from build123d import *

# Parameters (mm, degrees)
SKETCH2_W               = 6
SKETCH2_H               = 15
CUT_EXTRUDE1_DEPTH      = 45.71
CUT_EXTRUDE2_DEPTH      = 57.171431365
CUT_EXTRUDE2_DEPTH_BACK = 19
SKETCH4_R               = 3


with BuildPart() as part:
    # Model → Revolve1 (revolve)
    with BuildSketch(Plane.XY, mode=Mode.PRIVATE) as revolve1_sk:
        with BuildLine():
            Line((-27.291095715, -5.663546948), (-27.291095715, -10.663546948))
            Line((-27.291095715, -10.663546948), (-27.291095715, -51.373546948))
            ThreePointArc((-27.291095715, -51.373546948), (-28.755561809, -54.909080854), (-32.291095715, -56.373546948))
            Line((-32.291095715, -56.373546948), (-32.291095715, -52.264917369))
            Line((-32.291095715, -52.264917369), (-32.291095715, -10.663546948))
            Line((-32.291095715, -10.663546948), (-32.291095715, 35.040839423))
            Line((-32.291095715, 35.040839423), (-30.291095715, 35.040839423))
            Line((-30.291095715, 35.040839423), (-30.291095715, 26.12431753))
            Line((-30.291095715, 26.12431753), (-28.291095715, 26.12431753))
            Line((-28.291095715, 26.12431753), (-28.291095715, 5.494079969))
            Line((-28.291095715, 5.494079969), (-27.291095715, 5.494079969))
            Line((-27.291095715, 5.494079969), (-27.291095715, 2.336453052))
            Line((-27.291095715, 2.336453052), (-28.291095714, 2.336453052))
            Line((-28.291095714, 2.336453052), (-28.291095714, -5.663546948))
            Line((-28.291095714, -5.663546948), (-27.291095715, -5.663546948))
        make_face()
    revolve(revolve1_sk.sketch.rotate(Axis((-32.291095715, 35.040839423, 0), (0, 1, 0)), 90), axis=Axis((-32.291095715, 35.040839423, 0), (0, 1, 0)))

    # Sketch2 → Cut-Extrude1 (cut)
    with BuildSketch(Plane(origin=(0, -56.373546948, 0), x_dir=(-1, 0, 0), z_dir=(0, -1, 0))):
        with Locations((32.291095715, 1.617056414)):
            Rectangle(SKETCH2_W, SKETCH2_H)
    extrude(amount=-CUT_EXTRUDE1_DEPTH, mode=Mode.SUBTRACT)

    # Sketch4 → Cut-Extrude2 (cut, two sides: drawn at the far end of the back side and taken through both)
    with BuildSketch(Plane(origin=(-35.291095715, 0, 0), x_dir=(0, 0, -1), z_dir=(1, 0, 0)).offset(-CUT_EXTRUDE2_DEPTH_BACK)):
        with Locations(Location((0, -51.373546948, 0), (0, 0, 180))):
            Circle(SKETCH4_R)
    extrude(amount=CUT_EXTRUDE2_DEPTH + CUT_EXTRUDE2_DEPTH_BACK, mode=Mode.SUBTRACT)


solid = part.part
Verification items for the finished model (mm, model axes). A direction names the side the tool comes from. Round coordinates to 2 decimals unless told otherwise and drop trailing zeros. Loops run counter-clockwise (first coordinate to the right, second up) from the corner with the lowest first, then second, coordinate; pieces in that order, holes last. Notation, with made-up numbers: (-19.75, 27) - (12.25, 27) arc R27 ccw to (12.25, 64) - close; hole circle Ø8 at (59.5, 88). An arc over 180 degrees is marked (long way). Answer in a Markdown table with one row per item. Add a question column.
Q1. Section check B-B on y = 1. Enter the section's corners in (x, z), plus the area to 3 significant figures.
Q2. Release check for a two-part mould opening along Y. For faces 1 (the face through (-31, 26.124, -2)), 2 (the face through (-32, -10.664, 0)), 3 (the face through (-29.291, -33, 0)), 4 (the face through (-28.525, -48.445, -0.65)) record: pulls with the +Y half, pulls with the -Y half, needs draft (parallel to the pull), parting line crosses it, or undercut.
Q3. Gauge pin test, flat ends, axial feed: pin 1 (1.8 mm diameter, centred on x = -33.5, z = 1.5, fed in from -Y); pin 2 (2 mm diameter, centred on y = -11.5, z = -3.5, fed in from +X); pin 3 (1.5 mm diameter, centred on x = -31, y = -9, fed in from +Z). Record the tip position at first contact, or that the pin passes through.
Q4. Material ranges on line 1 (Y direction, x = -27.7, z = 0); line 2 (Y direction, x = -35, z = 3); line 3 (X direction, y = -20.5, z = 0.25), recorded low to high.
Q5. Section check A-A on z = 0. State how many separate pieces and enclosed holes the cut face has, plus the area to 3 significant figures.
Q6. Tool access check on faces 5 (the face through (-32, 35.041, 0)), 6 (the face through (-35.291, -33, 0)), 7 (the face through (-36, 2.336, 2)), 8 (the face through (-34.274, 30.52, 0.26)), 9 (the face through (-35.67, -28.839, 3.685)). Record the directions out of +Z, -Z, +X, -X, +Y, -Y that give a thin tool (end or side, any length) a straight path to the whole face; none if there is none.
Q7. Section check C-C on y = 27.5. Enter the section's corners in (x, z), plus the area to 3 significant figures.
Found:
| question | item | result |
|---|---|---|
| 1 | outline | circle Ø8 at (-32.29, 0) |
| 1 | area | 50.3 mm² |
| 2 | face 1 | pulls with the +Y half |
| 2 | face 2 | pulls with the -Y half |
| 2 | face 3 | needs draft |
| 2 | face 4 | undercut |
| 3 | pin 1 | stops at y = -10.66 |
| 3 | pin 2 | stops at x = -27.96 |
| 3 | pin 3 | stops at z = 4.97 |
| 4 | line 1 | y = -48.37 to -5.66, 2.34 to 5.49 |
| 4 | line 2 | y = -10.66 to -5.66, 2.34 to 5.49 |
| 4 | line 3 | x = -37.28 to -35.29, -29.29 to -27.3 |
| 5 | separate pieces | 3 |
| 5 | enclosed holes | 0 |
| 5 | area | 498 mm² |
| 6 | face 5 | +Z, -Z, +X, -X, +Y |
| 6 | face 6 | +Z, -Z, -Y |
| 6 | face 7 | none |
| 6 | face 8 | +Y |
| 6 | face 9 | +Y, -Y |
| 7 | outline | circle Ø4 at (-32.29, 0) |
| 7 | area | 12.6 mm² |
